Read the model definition and answer for the solid it produces. Units are mm, in the model's axes. A direction names the side the tool comes from. Coordinates: 2 decimals unless noted, no trailing zeros. Write each loop counter-clockwise with the first axis right and the second up, starting at its lowest first coordinate (ties: lowest second). Pieces come first, ordered by that corner, then holes.
(1) Which of the six approach directions +Z, -Z, +X, -X, +Y, -Y give full straight-line access (tool end or side, diameter ignored) to faces 4 (the cylindrical face through (3.864, 20.914, -17.252)), 5 (the flat face through (0, 0, 0)), 6 (the flat face through (11, 19.05, -15))?
(2) The part is cut by section A-A, the plane x = 22. Determine the outline of the cut face in (y, z) (3 decimals), and give its area (3 significant figures).
(3) Determine the mould class of faces 1 (the flat face through (25.4, -5, 0)), 2 (the flat face through (0, -19.05, 0)), 3 (the conical face through (0.012, 23.335, -17.74)) for opening direction X: pulls with the +X half, pulls with the -X half, needs draft (parallel to the pull), parting line crosses it, or undercut.
(4) Given pin 1 (7.5 mm diameter, centred on x = 0, y = 15.875, fed in from -Z); pin 2 (2.5 mm diameter, centred on x = 0, z = -17.46, fed in from +Y); pin 3 (5 mm diameter, centred on x = -12.7, z = -17.46, fed in from +Y); pin 4 (5 mm diameter, centred on x = 12.5, z = -17.5, fed in from +Y), each flat-ended and moving along its own axis, determine where each tip first touches the part or whether it passes through.
(5) Straight lines are drawn through the part: line 1 along Z through (x, y) = (-12.7, 26.5) (1 decimal); line 2 along Z through (x, y) = (3.5, 22) (3 decimals); line 3 along Z through (x, y) = (12.7, 17.05) (3 decimals). For each, find the intervals that lie inside material, in ascending order.
(6) The part is cut by section B-B, the plane y = 14. State how many separate pieces and enclosed holes the cut face has, and give its area (3 significant figures).
```python
from build123d import *

# Parameters (mm, degrees)
BASE_BLOCK_DEPTH         = 25.4
DOWEL_HOLE_0_126IN_D     = 3.2004
DOWEL_HOLE_0_126IN_DEPTH = 7.62
DOWEL_HOLE_0_126IN_TIP   = 0.961497163
DOWEL_HOLE_CHAMFER_SIZE  = 1.27
BORE_0_5IN_THRU_D        = 12.7
BORE_EDGE_CHAMFER_SIZE   = 0.635


with BuildPart() as part:
    # Base Block Profile Sketch → Base Block (new, symmetric)
    with BuildSketch(Plane(origin=(0, 0, 0), x_dir=(0, 0, -1), z_dir=(1, 0, 0))):
        Polygon((-9.525, 0), (9.525, 0), (9.525, 31.75), (25.4, 31.75), (25.4, 0), (25.4, -19.05), (-25.4, -19.05), (-25.4, 0), (-25.4, 31.75), (-9.525, 31.75), align=None)
    extrude(amount=BASE_BLOCK_DEPTH, both=True)

    # Dowel Hole 0.126in
    with Locations(Plane(origin=(0, 31.75, -17.4625), x_dir=(0, 0, 1), z_dir=(0, 1, 0))):
        with Locations((0, 0)):
            Hole(DOWEL_HOLE_0_126IN_D / 2, depth=DOWEL_HOLE_0_126IN_DEPTH)
            with Locations((0, 0, -(DOWEL_HOLE_0_126IN_DEPTH + DOWEL_HOLE_0_126IN_TIP / 2))):  # 118° drill point
                Cone(0, DOWEL_HOLE_0_126IN_D / 2, DOWEL_HOLE_0_126IN_TIP, mode=Mode.SUBTRACT)

    # Dowel Hole Chamfer
    dowel_hole_chamfer_edges = [part.edges().sort_by_distance(p)[0] for p in [
        (0, 31.75, -15.8623),
    ]]
    chamfer(dowel_hole_chamfer_edges, length=DOWEL_HOLE_CHAMFER_SIZE)

    # Sketch5 → Tapped Hole M-quarter-20 A (revolve, cut)
    with BuildSketch(Plane(origin=(12.7, 31.75, -17.4625), x_dir=(0, 0, 1), z_dir=(1, 0, 0))):
        Polygon((0, 0), (0, 19.0627), (2.5527, 16.51), (2.5527, 12.7), (3.175, 12.7), (3.175, 0.730483939), (3.81, 0), align=None)
    revolve(axis=Axis((12.7, 38.1, -17.4625), (0, -1, 0)), mode=Mode.SUBTRACT)

    # Sketch6 → Tapped Hole M-quarter-20 B (revolve, cut)
    with BuildSketch(Plane(origin=(-12.7, 31.75, -17.4625), x_dir=(0, 0, 1), z_dir=(1, 0, 0))):
        Polygon((0, 0), (0, 19.0627), (2.5527, 16.51), (2.5527, 12.7), (3.175, 12.7), (3.175, 0.876580726), (3.937, 0), align=None)
    revolve(axis=Axis((-12.7, 38.1, -17.4625), (0, -1, 0)), mode=Mode.SUBTRACT)

    # Bore 0.5in Thru (through all)
    with Locations(Plane(origin=(0, 15.875, 25.4), x_dir=(0, 1, 0), z_dir=(0, 0, 1))):
        with Locations((0, 0)):
            Hole(BORE_0_5IN_THRU_D / 2)

    # Bore Edge Chamfer
    bore_edge_chamfer_edges = [part.edges().sort_by_distance(p)[0] for p in [
        (0, 22.225, -25.4),
        (0, 22.225, 25.4),
    ]]
    chamfer(bore_edge_chamfer_edges, length=BORE_EDGE_CHAMFER_SIZE)


solid = part.part
```
Computed:
1. face 4: +Z, -Z
1. face 5: +X, -X, +Y
1. face 6: +Y
2. outline: (-19.05, -25.4) - (31.75, -25.4) - (31.75, -9.525) - (0, -9.525) - (0, 9.525) - (31.75, 9.525) - (31.75, 25.4) - (-19.05, 25.4) - close
2. area: 1,980 mm2
3. face 1: pulls with the +X half
3. face 2: needs draft
3. face 3: undercut
4. pin 1: passes through
4. pin 2: stops at y = 23.92
4. pin 3: stops at y = 15.19
4. pin 4: stops at y = 19.05
5. line 1: z = -25.4 to -20.6, -14.3 to -9.5, 9.5 to 25.4
5. line 2: z = -25.4 to -9.525, 9.525 to 25.4
5. line 3: z = -25.4 to -20.015, -14.91 to -9.525, 9.525 to 25.4
6. separate pieces: 4
6. enclosed holes: 2
6. area: 1,220 mm2
